Part print with two shaded views. Sizes in mm from the minimum x, y, z corner. Round coordinates to 2 decimals unless told otherwise and drop trailing zeros. Answer as a JSON object with one key per item and string values.
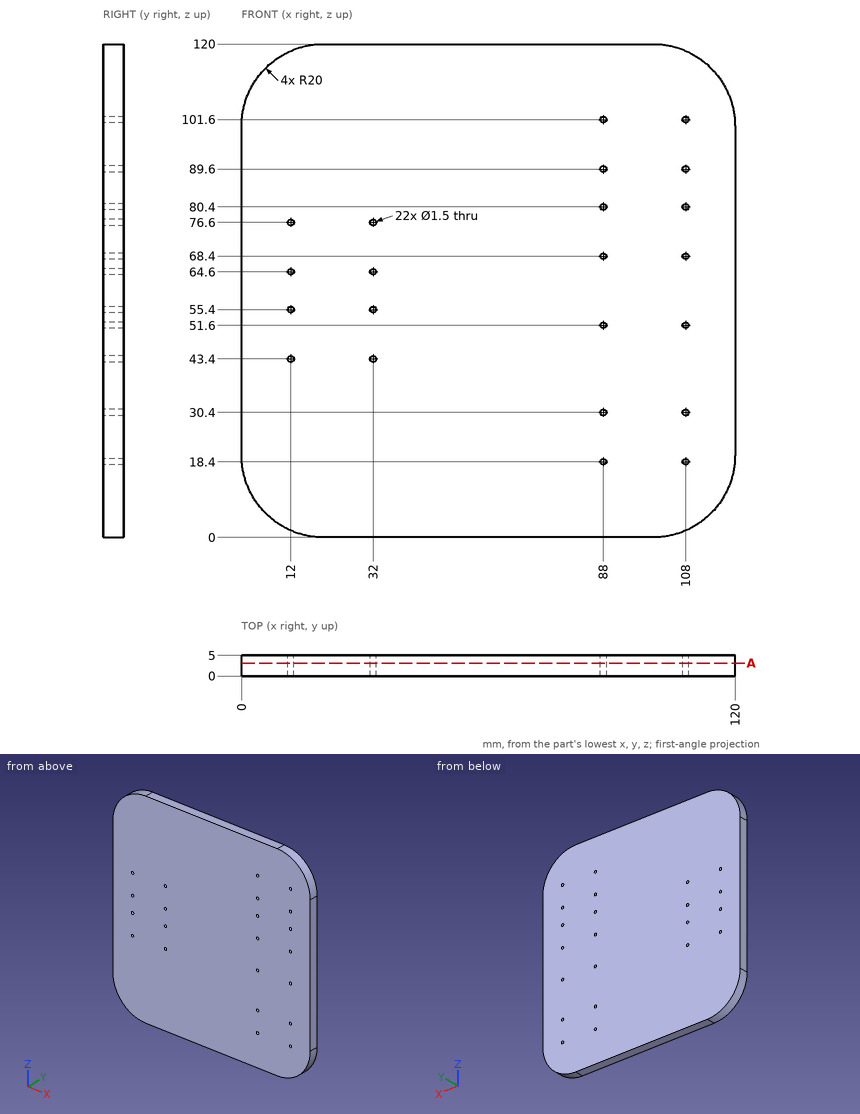
Item 1: Wall check: line 1 along X through (y, z) = (1.65, 43.4); line 2 along X through (y, z) = (3.4, 89.6); line 3 along Z through (x, y) = (31.5, 1.7). Give the ranges that are in metal, low to high. Write a range as [from, to].
Worked answers:
{"line 1": "x = [0, 11.25], [12.75, 31.25], [32.75, 120]", "line 2": "x = [0, 87.25], [88.75, 107.25], [108.75, 120]", "line 3": "z = [0, 42.84], [43.96, 54.84], [55.96, 64.04], [65.16, 76.04], [77.16, 120]"}
Item 2: Drop a flat-ended pin along its axis: pin 1 Ø1.2 at (x, z) = (88, 89.6) entering from -Y. Give the stop position or say it passes through.
Worked answers:
{"pin 1": "passes through"}
Item 3: Saw through at A-A on y = 3.15. State how many separate pieces and enclosed holes the cut face has, and give its area (3 significant figures).
Worked answers:
{"separate pieces": "1", "enclosed holes": "22", "area": "14,000 mm2"}
